Design review of the part built by this model. Coordinates are the model's own, in mm. Face numbers are marked on the shaded views. A direction names the side the tool comes from. Give positions to 0.01 mm unless a question says otherwise; leave off trailing zeros. Write each loop counter-clockwise with the first axis right and the second up, starting at its lowest first coordinate (ties: lowest second). Pieces come first, ordered by that corner, then holes. Notation, with made-up numbers: M -32.5,39.25 L 8.5,39.25 A20 cw 8.5,53.25 Z; hole C -23,-4 d3. An arc over 180 degrees is marked long. Use one line per item in the form item = value. Start each with the question number.
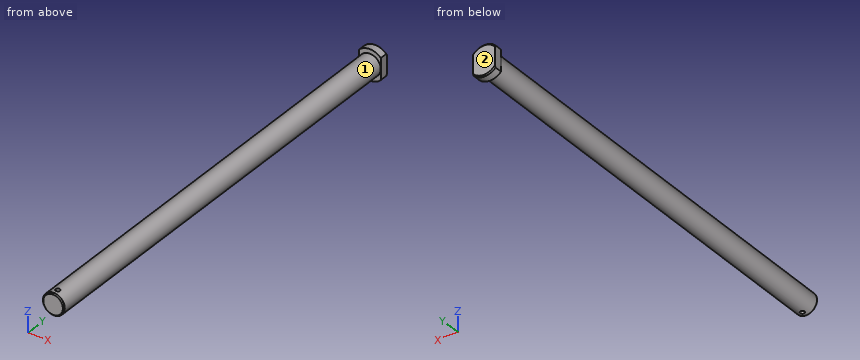
from build123d import *

# Parameters (mm, degrees)
CHAMFER1_SIZE           = 0.5
CUT_EXTRUDE1_DEPTH      = 208.236579783
CUT_EXTRUDE1_DEPTH_BACK = 208.236579783
SKETCH2_R               = 1
CUT_EXTRUDE2_DEPTH      = 208.236579783
CUT_EXTRUDE2_DEPTH_BACK = 208.236579783
SKETCH3_W               = 2
SKETCH3_H               = 4
CUT_EXTRUDE3_DEPTH      = 208.236579783
CUT_EXTRUDE3_DEPTH_BACK = 208.236579783
SKETCH4_W               = 2
SKETCH4_H               = 4


with BuildPart() as part:
    # Sketch1 → Revolve1 (revolve)
    with BuildSketch(Plane.XY):
        Polygon((0, 0), (7, 0), (7, -4), (5, -4), (5, -207), (0, -207), align=None)
    revolve(axis=Axis((0, -318.988143723, 0), (0, 1, 0)))

    # Chamfer1
    chamfer1_edges = [part.edges().sort_by_distance(p)[0] for p in [
        (-5, -207, 0),
        (-7, 0, 0),
    ]]
    chamfer(chamfer1_edges, length=CHAMFER1_SIZE)

    # Sketch2 → Cut-Extrude1 (cut, two sides: drawn at the far end of the back side and taken through both)
    with BuildSketch(Plane.XY.offset(-CUT_EXTRUDE1_DEPTH_BACK)):
        with Locations((0, -204)):
            Circle(SKETCH2_R)
    extrude(amount=CUT_EXTRUDE1_DEPTH + CUT_EXTRUDE1_DEPTH_BACK, mode=Mode.SUBTRACT)

    # Sketch3 → Cut-Extrude2 (cut, two sides: drawn at the far end of the back side and taken through both)
    with BuildSketch(Plane.XY.offset(-CUT_EXTRUDE2_DEPTH_BACK)):
        with Locations((-6, -2)):
            Rectangle(SKETCH3_W, SKETCH3_H)
    extrude(amount=CUT_EXTRUDE2_DEPTH + CUT_EXTRUDE2_DEPTH_BACK, mode=Mode.SUBTRACT)

    # Sketch4 → Cut-Extrude3 (cut, two sides: drawn at the far end of the back side and taken through both)
    with BuildSketch(Plane.XY.offset(-CUT_EXTRUDE3_DEPTH_BACK)):
        with Locations((6, -2)):
            Rectangle(SKETCH4_W, SKETCH4_H)
    extrude(amount=CUT_EXTRUDE3_DEPTH + CUT_EXTRUDE3_DEPTH_BACK, mode=Mode.SUBTRACT)


solid = part.part
1. Clearance check with flat-ended pins moving along their axes: pin 1 Ø6 at (x, y) = (2, -104.5) entering from -Z; pin 2 Ø2 at (x, y) = (1.5, -133) entering from +Z; pin 3 Ø1.8 at (x, y) = (0, -204) entering from +Z; pin 4 Ø3 at (y, z) = (-132.5, -3) entering from +X. State where each tip first meets the part, or that it passes through.
2. To check wall thickness, follow L1, parallel to X at y = -204, z = -1; L2, parallel to X at y = -204, z = -0.25; L3, parallel to Y at x = 4, z = 4.25. State the ranges of each line that lie inside material, in increasing order.
3. We need section A-A (y = -125). State the section outline as (x, z) points, and give its area (3 significant figures).
4. For the marked faces 1 and 2, list the 3-axis set-ups (+Z, -Z, +X, -X, +Y, -Y) from which the entire face can be reached by the end or side of a thin tool; tool diameter is ignored.
Answer block:
q1.pin_1 = -5
q1.pin_2 = 4.97
q1.pin_3 = through
q1.pin_4 = 4.77
q2.L1 = -4.9 to -1, 1 to 4.9
q2.L2 = -4.99 to -1, 1 to 4.99
q2.L3 = -4 to 0
q3.outline = C 0,0 d10
q3.area = 78.5 mm^2
q4.face_1 = -Y
q4.face_2 = +Z, -Z, +X, -X, +Y
